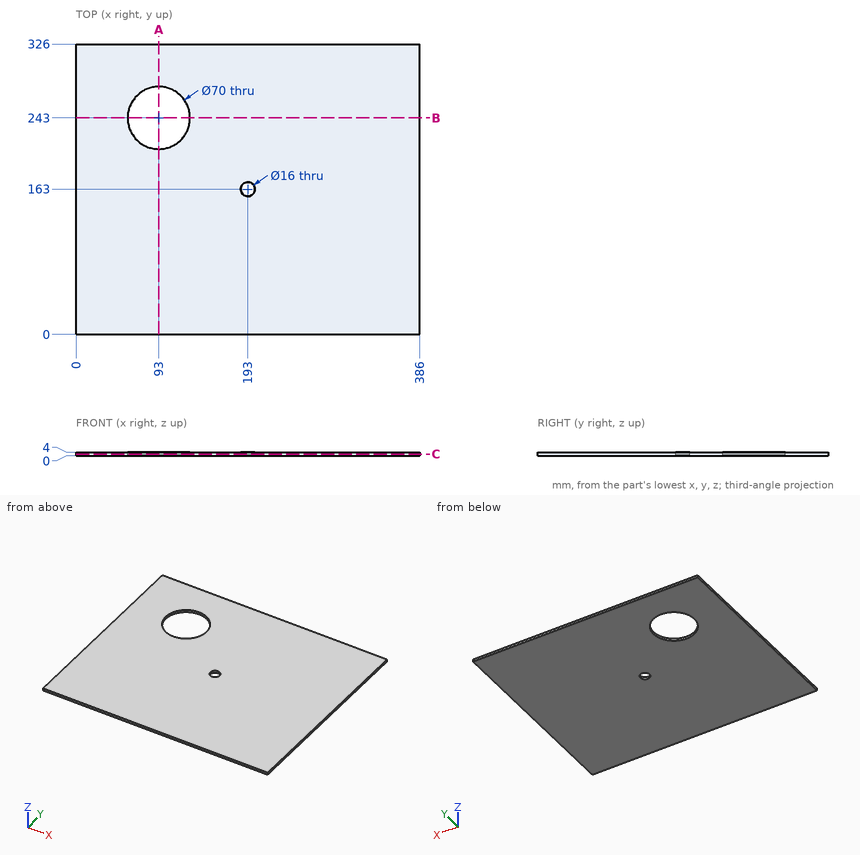
Print and shaded views of the part. All mm, measured from the part's lowest x, y and z. Give positions to 0.01 mm unless a question says otherwise; leave off trailing zeros. Loops run counter-clockwise (first coordinate to the right, second up) from the corner with the lowest first, then second, coordinate; pieces in that order, holes last. Notation, with made-up numbers: M 85,86.5 L 139,86.5 A18 ccw 139,102.5 Z; hole C -26.5,-17 d9. An arc over 180 degrees is marked long. Write each question's results on one line, items separated by ' | '.
Q1. Band-saw the part on C-C on z = 1.8. Write the cut outline in (x, y).
Geometry check:
outline: M 0,0 L 386,0 L 386,326 L 0,326 Z; hole C 93,243 d70; hole C 193,163 d16
Q2. Band-saw the part on A-A on x = 93. Write the cut outline in (y, z), and give its area (3 significant figures).
Geometry check:
outline: M 0,0 L 208,0 L 208,4 L 0,4 Z; M 278,0 L 326,0 L 326,4 L 278,4 Z | area: 1,020 mm²
Q3. Band-saw the part on B-B on y = 243. Write the cut outline in (x, z), and give its area (3 significant figures).
Geometry check:
outline: M 0,0 L 58,0 L 58,4 L 0,4 Z; M 128,0 L 386,0 L 386,4 L 128,4 Z | area: 1,260 mm²
Q4. Flat gauge pin, fed straight in: P1, Ø14.5, axis at x = 193, y = 163, coming from the -Z side. Where does the tip first touch, or does it go through?
Geometry check:
P1: passes through
Q5. Probe probe 1 along Y at (x, z) = (93, 3.05); probe 2 along Y at (x, z) = (193, 2.05); probe 3 along X at (y, z) = (163, 3.1). List the from-to ranges inside material, lowest first.
Geometry check:
probe 1: y = 0 to 208, 278 to 326 | probe 2: y = 0 to 155, 171 to 326 | probe 3: x = 0 to 185, 201 to 386
